Geometry check sheet. Reference: the model listing, model coordinates, mm. Coordinates: 2 decimals unless noted, no trailing zeros. Write each loop counter-clockwise with the first axis right and the second up, starting at its lowest first coordinate (ties: lowest second). Pieces come first, ordered by that corner, then holes. Notation, with made-up numbers: (-37.5, 48) -> (-4.5, 48) arc R22 ccw to (-4.5, 55) -> close; hole circle Ø4 at (-8, 62). An arc over 180 degrees is marked (long way). Answer in a Markdown table with one row per item. Add a question column.
Q1. Section check C-C, the plane z = -5.5. Record the boundary of the cut face in (x, y), and give its area (3 significant figures).
Q2. Thickness scan on line 1 (Y direction, x = 75, z = -3.5); line 2 (Y direction, x = -67, z = 2.25); line 3 (X direction, y = 78.5, z = 3.75). Record the ranges inside material, lowest first.
Q3. Release check for a two-part mould opening along Y. For faces 1 (the face through (-1, -100, 0)), 2 (the face through (-100, -1, 0)), 3 (the face through (67.261, -67.904, 0.112)) record: pulls with the +Y half, pulls with the -Y half, needs draft (parallel to the pull), parting line crosses it, or undercut.
Q4. Gauge pin test, flat end, axial feed: P1, Ø19, axis at x = -75, y = -75, coming from the +Z side. Record the tip position at first contact, or that the pin passes through.
Q5. Section check A-A, the plane y = 75. Record the boundary of the cut face in (x, z).
```python
from build123d import *

# Parameters (mm, degrees)
SKETCH1_W      = 200
SKETCH1_H      = 200
EXTRUDE1_DEPTH = 8
SKETCH2_R      = 10.5
EXTRUDE2_DEPTH = 143.323574997


with BuildPart() as part:
    # Sketch1 → Extrude1 (new, symmetric)
    with BuildSketch(Plane.XY):
        Rectangle(SKETCH1_W, SKETCH1_H)
    extrude(amount=EXTRUDE1_DEPTH, both=True)

    # Sketch2 → Extrude2 (cut, through all)
    with BuildSketch(Plane.XY.offset(8)):
        with Locations((-75, 75)):
            Circle(SKETCH2_R)
        with Locations((75, 75)):
            Circle(SKETCH2_R)
        with Locations((-75, -75)):
            Circle(SKETCH2_R)
        with Locations((75, -75)):
            Circle(SKETCH2_R)
    extrude(amount=-EXTRUDE2_DEPTH, mode=Mode.SUBTRACT)


solid = part.part
```
Calculated:
| question | item | result |
|---|---|---|
| 1 | outline | (-100, -100) -> (100, -100) -> (100, 100) -> (-100, 100) -> close; hole circle Ø21 at (-75, -75); hole circle Ø21 at (-75, 75); hole circle Ø21 at (75, -75); hole circle Ø21 at (75, 75) |
| 1 | area | 38,600 mm² |
| 2 | line 1 | y = -100 to -85.5, -64.5 to 64.5, 85.5 to 100 |
| 2 | line 2 | y = -100 to -81.8, -68.2 to 68.2, 81.8 to 100 |
| 2 | line 3 | x = -100 to -84.9, -65.1 to 65.1, 84.9 to 100 |
| 3 | face 1 | pulls with the -Y half |
| 3 | face 2 | needs draft |
| 3 | face 3 | undercut |
| 4 | P1 | passes through |
| 5 | outline | (-100, -8) -> (-85.5, -8) -> (-85.5, 8) -> (-100, 8) -> close; (-64.5, -8) -> (64.5, -8) -> (64.5, 8) -> (-64.5, 8) -> close; (85.5, -8) -> (100, -8) -> (100, 8) -> (85.5, 8) -> close |
